```python
from build123d import *

# Parameters (mm, degrees)
SKETCH_1_W           = 30
SKETCH_1_H           = 45
BOSS_EXTRUDE_1_DEPTH = 7
CUT_EXTRUDE_1_DEPTH  = 28.932955447
M6_TAPPED_HOLE_1_D   = 5


with BuildPart() as part:
    # Sketch 1 → Boss-Extrude 1 (new body)
    with BuildSketch(Plane.XY):
        Rectangle(SKETCH_1_W, SKETCH_1_H)
    extrude(amount=BOSS_EXTRUDE_1_DEPTH)

    # Sketch 2 → Cut-Extrude 1 (cut, through all)
    with BuildSketch(Plane(origin=(0, 0, 0), x_dir=(-1, 0, 0), z_dir=(0, 0, -1))):
        with BuildLine():
            Line((10, 15.75), (-10, 15.75))
            ThreePointArc((-10, 15.75), (-11.75, 17.5), (-10, 19.25))
            Line((-10, 19.25), (10, 19.25))
            ThreePointArc((10, 19.25), (11.75, 17.5), (10, 15.75))
        make_face()
    extrude(amount=-CUT_EXTRUDE_1_DEPTH, mode=Mode.SUBTRACT)

    # M6 Tapped Hole 1 (through all)
    with Locations(Plane(origin=(0, 0, 0), x_dir=(-1, 0, 0), z_dir=(0, 0, -1))):
        with Locations((7, -15.5), (-7, -5.5)):
            Hole(M6_TAPPED_HOLE_1_D / 2)


solid = part.part
```
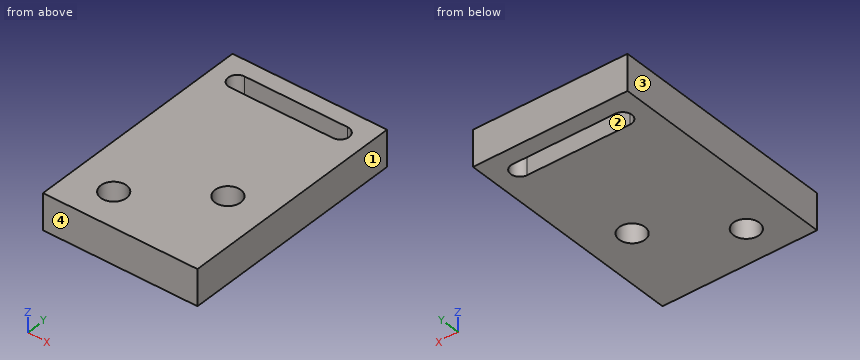
Work out the finished part from the listing and answer in its coordinate system (mm). Face numbers are marked on the shaded views. Coordinates: 2 decimals unless noted, no trailing zeros. Loops run counter-clockwise (first coordinate to the right, second up) from the corner with the lowest first, then second, coordinate; pieces in that order, holes last.
1) Consider probe 1 along Y at (x, z) = (-7, 5); probe 2 along Y at (x, z) = (7, 4.75); probe 3 along Y at (x, z) = (0, 2.5). Determine where each line is inside the solid, lowest interval first.
Results:
probe 1: y = -22.5 to -18, -13 to 15.75, 19.25 to 22.5
probe 2: y = -22.5 to -8, -3 to 15.75, 19.25 to 22.5
probe 3: y = -22.5 to 15.75, 19.25 to 22.5
2) Section B-B (y = -15.5) is taken. Give the vertices of the cut face in (x, z).
Results:
outline: (-15, 0) - (-9.5, 0) - (-9.5, 7) - (-15, 7) - close; (-4.5, 0) - (15, 0) - (15, 7) - (-4.5, 7) - close
3) Section D-D (x = 2) is taken. Give the vertices of the cut face in (y, z).
Results:
outline: (-22.5, 0) - (15.75, 0) - (15.75, 7) - (-22.5, 7) - close; (19.25, 0) - (22.5, 0) - (22.5, 7) - (19.25, 7) - close
4) Section C-C (z = 4.5) is taken. Give the vertices of the cut face in (x, y), plus the area to 3 significant figures.
Results:
outline: (-15, -22.5) - (15, -22.5) - (15, 22.5) - (-15, 22.5) - close; hole (-10, 15.75) - (10, 15.75) arc R1.75 ccw to (10, 19.25) - (-10, 19.25) arc R1.75 ccw to start; hole circle Ø5 at (-7, -15.5); hole circle Ø5 at (7, -5.5)
area: 1,230 mm2
5) Section A-A (x = -7) is taken. Give the vertices of the cut face in (y, z).
Results:
outline: (-22.5, 0) - (-18, 0) - (-18, 7) - (-22.5, 7) - close; (-13, 0) - (15.75, 0) - (15.75, 7) - (-13, 7) - close; (19.25, 0) - (22.5, 0) - (22.5, 7) - (19.25, 7) - close
6) For a pull along X with two mould halves and no side action, classify the marked faces 1, 2, 3 and 4 as +X half, -X half, draft (parallel to the pull), parting line (faces both ways), or undercut.
Results:
face 1: +X half
face 2: undercut
face 3: -X half
face 4: draft
